Read the model definition and answer for the solid it produces. Units are mm, in the model's axes. Coordinates: 2 decimals unless noted, no trailing zeros. Loops run counter-clockwise (first coordinate to the right, second up) from the corner with the lowest first, then second, coordinate; pieces in that order, holes last. Notation, with made-up numbers: M -11.5,-30.5 L 9.5,-30.5 A27 ccw 9.5,3.5 Z; hole C 71.25,82.5 d3. An arc over 180 degrees is marked long. Use one line per item in the form item = value. Start each with the question number.
1. Find the intervals of material crossed by probe 1 along Y at (x, z) = (-66.5, 10.75); probe 2 along X at (y, z) = (-134.5, 5.75); probe 3 along Y at (x, z) = (-11, 1.5), in increasing order. Write a range as [from, to].
2. The part is cut by section A-A (y = -72). Give the vertices of the cut face in (x, z).
3. Flat-ended cylindrical pins translate along their axes: pin 1 (4 mm diameter, centred on x = -20.5, z = 9, fed in from -Y); pin 2 (2 mm diameter, centred on x = -54.5, z = 5.5, fed in from -Y). Find the tip coordinate at first contact, or state that the pin passes through.
4. The part is cut by section B-B (x = -66). Give the vertices of the cut face in (y, z).
5. The part is cut by section C-C (z = 6.25). Give the vertices of the cut face in (x, y), plus the area to 3 significant figures.
6. The part is cut by section D-D (y = -12). Give the vertices of the cut face in (x, z).
7. For a pull along X with two mould halves and no side action, classify faces 1 (the flat face through (-56, -63, 0)), 2 (the cylindrical face through (-70.5, -10.47, 7.39)), 3 (the cylindrical face through (-64.971, -66.943, 7.395)), 4 (the flat face through (-90.635, -81, 7)) as released by +X, released by -X, zero draft, split by the parting line, or undercut.
from build123d import *

# Parameters (mm, degrees)
SKETCH1_R              = 4.5
BOSS_EXTRUDE2_DEPTH    = 15
M12_TAPPED_HOLE1_D     = 10.2
M12_TAPPED_HOLE1_DEPTH = 29.25
M12_TAPPED_HOLE1_TIP   = 3.064389157


with BuildPart() as part:
    # Sketch1 → Boss-Extrude2 (new body)
    with BuildSketch(Plane.XY):
        Polygon((0, 0), (-90.634528925, 0), (-90.634528925, -165), align=None)
        with Locations((-65.634528925, -12)):
            Circle(SKETCH1_R, mode=Mode.SUBTRACT)
        with Locations((-65.634528925, -72)):
            Circle(SKETCH1_R, mode=Mode.SUBTRACT)
    extrude(amount=BOSS_EXTRUDE2_DEPTH)

    # M12 Tapped Hole1
    with Locations(Plane.XY.offset(15)):
        with Locations((-65.634528925, -12), (-65.634528925, -72)):
            Hole(M12_TAPPED_HOLE1_D / 2, depth=M12_TAPPED_HOLE1_DEPTH)
            with Locations((0, 0, -(M12_TAPPED_HOLE1_DEPTH + M12_TAPPED_HOLE1_TIP / 2))):  # 118° drill point
                Cone(0, M12_TAPPED_HOLE1_D / 2, M12_TAPPED_HOLE1_TIP, mode=Mode.SUBTRACT)


solid = part.part
Computed values:
q1.probe_1 = [-121.06, -77.03], [-66.97, -17.03], [-6.97, 0]
q1.probe_2 = [-90.63, -73.88]
q1.probe_3 = [-20.03, 0]
q2.outline = M -90.63,0 L -70.73,0 L -70.73,15 L -90.63,15 Z; M -60.53,0 L -39.55,0 L -39.55,15 L -60.53,15 Z
q3.pin_1 = -40.96
q3.pin_2 = -101.04
q4.outline = M -120.15,0 L -77.09,0 L -77.09,15 L -120.15,15 Z; M -66.91,0 L -17.09,0 L -17.09,15 L -66.91,15 Z; M -6.91,0 L 0,0 L 0,15 L -6.91,15 Z
q5.outline = M -90.63,-165 L 0,0 L -90.63,0 Z; hole C -65.63,-72 d10.2; hole C -65.63,-12 d10.2
q5.area = 7,310 mm²
q6.outline = M -90.63,0 L -70.73,0 L -70.73,15 L -90.63,15 Z; M -60.53,0 L -6.59,0 L -6.59,15 L -60.53,15 Z
q7.face_1 = zero draft
q7.face_2 = undercut
q7.face_3 = undercut
q7.face_4 = released by -X
